Geometry check sheet. Reference: the model listing, model coordinates, mm. Face numbers are marked on the shaded views. A direction names the side the tool comes from. Give positions to 0.01 mm unless a question says otherwise; leave off trailing zeros. Loops run counter-clockwise (first coordinate to the right, second up) from the corner with the lowest first, then second, coordinate; pieces in that order, holes last. Notation, with made-up numbers: (-4, 44) -> (32, 44) arc R23 cw to (32, 83) -> close; hole circle Ø7 at (0.25, -25). An arc over 180 degrees is marked (long way). Answer as a JSON object with one key per item and string values.
from build123d import *

# Parameters (mm, degrees)
EXTRUDE_1_DEPTH     = 7.5
CUT_EXTRUDE_1_REACH = 49.762
SKETCH_2_R          = 2


with BuildPart() as part:
    # 草图1 → 凸台-拉伸1 (new, symmetric)
    with BuildSketch(Plane.XY):
        Polygon((0, 0), (47, 0), (47, 4), (39, 4), (39, 2), (0, 2), align=None)
    extrude(amount=EXTRUDE_1_DEPTH, both=True)

    # 草图2 → 切除-拉伸1 (cut, up to next)
    with BuildSketch(Plane(origin=(0, 4, 0), x_dir=(1, 0, 0), z_dir=(0, 1, 0)), mode=Mode.PRIVATE) as cut_extrude_1_sk1:
        with Locations(Location((43, 3.5, 0), (0, 0, 180))):
            Circle(SKETCH_2_R)
    cut_extrude_1_tool1 = extrude(cut_extrude_1_sk1.sketch, amount=-CUT_EXTRUDE_1_REACH, mode=Mode.PRIVATE) & part.part
    # 草图2 → 切除-拉伸1 (cut, up to next)
    with BuildSketch(Plane(origin=(0, 4, 0), x_dir=(1, 0, 0), z_dir=(0, 1, 0)), mode=Mode.PRIVATE) as cut_extrude_1_sk2:
        with Locations(Location((43, -3.5, 0), (0, 0, 180))):
            Circle(SKETCH_2_R)
    cut_extrude_1_tool2 = extrude(cut_extrude_1_sk2.sketch, amount=-CUT_EXTRUDE_1_REACH, mode=Mode.PRIVATE) & part.part
    add(cut_extrude_1_tool1.solids().sort_by_distance((43, 4, -3.5))[0], mode=Mode.SUBTRACT)
    add(cut_extrude_1_tool2.solids().sort_by_distance((43, 4, 3.5))[0], mode=Mode.SUBTRACT)


solid = part.part
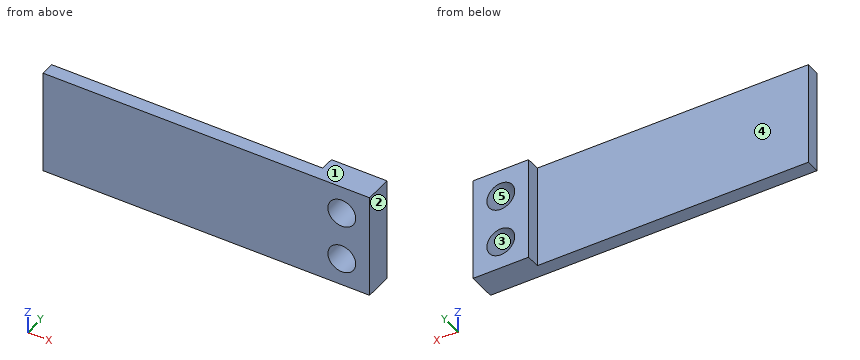
1) Depth check by flat-ended pin: P1, Ø1.6, axis at y = 3, z = -3, coming from the -X side; P2, Ø7.5, axis at x = 12, z = 2.5, coming from the +Y side. Enter the tip coordinate at first touch or a pass-through.
Geometry check:
{"P1": "stops at x = 39", "P2": "stops at y = 2"}
2) Section check D-D on x = 23.5. Record the cut outline in (y, z).
Geometry check:
{"outline": "(0, -7.5) -> (2, -7.5) -> (2, 7.5) -> (0, 7.5) -> close"}
3) Section check A-A on x = 43. Record the cut outline in (y, z).
Geometry check:
{"outline": "(0, -7.5) -> (4, -7.5) -> (4, -5.5) -> (0, -5.5) -> close; (0, -1.5) -> (4, -1.5) -> (4, 1.5) -> (0, 1.5) -> close; (0, 5.5) -> (4, 5.5) -> (4, 7.5) -> (0, 7.5) -> close"}
4) Section check B-B on z = -3.5. Record the cut outline in (x, y), plus the area to 3 significant figures.
Geometry check:
{"outline": "(0, 0) -> (41, 0) -> (41, 4) -> (39, 4) -> (39, 2) -> (0, 2) -> close; (45, 0) -> (47, 0) -> (47, 4) -> (45, 4) -> close", "area": "94.0 mm2"}
5) Material ranges on line 1 along Z through (x, y) = (43, 2.3); line 2 along Y through (x, z) = (6.5, 1); line 3 along X through (y, z) = (2.6, 5.75), recorded low to high. Write a range as from..to.
Geometry check:
{"line 1": "z = -7.5..-5.5, -1.5..1.5, 5.5..7.5", "line 2": "y = 0..2", "line 3": "x = 39..47"}
6) Section check C-C on y = 1.15. Record the cut outline in (x, z), plus the area to 3 significant figures.
Geometry check:
{"outline": "(0, -7.5) -> (47, -7.5) -> (47, 7.5) -> (0, 7.5) -> close; hole circle Ø4 at (43, -3.5); hole circle Ø4 at (43, 3.5)", "area": "680 mm2"}
7) Draft check along X on the marked faces 1, 2 and 3. Enter one of: pulls with the +X half, pulls with the -X half, needs draft (parallel to the pull), parting line crosses it, or undercut.
Geometry check:
{"face 1": "needs draft", "face 2": "pulls with the +X half", "face 3": "undercut"}
8) Tool access check on the marked faces 4 and 5. Record the directions out of +Z, -Z, +X, -X, +Y, -Y that give a thin tool (end or side, any length) a straight path to the whole face; none if there is none.
Geometry check:
{"face 4": "+Z, -Z, -X, +Y", "face 5": "+Y, -Y"}
